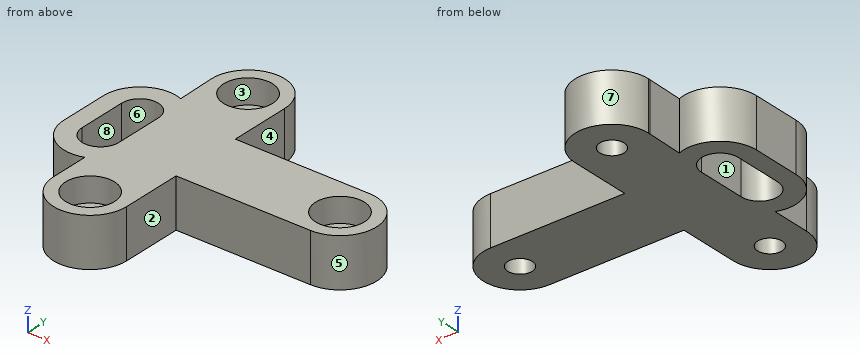
```python
from build123d import *

# Parameters (mm, degrees)
T_BRACKET_PLATE_20MM_DEPTH     = 20
POCKET_A_SKETCH_R              = 10
TRIANGULAR_POCKET_A_10MM_DEPTH = 10
POCKET_B_SKETCH_R              = 5
TRIANGULAR_POCKET_B_10MM_DEPTH = 10


with BuildPart() as part:
    # T Profile Sketch → T Bracket Plate 20mm (new body)
    with BuildSketch(Plane.XY):
        with BuildLine():
            ThreePointArc((-14.647668653, 24.012585384), (-28.506322055, 22.354856741), (-35, 10))
            Line((-35, 10), (-35, -10))
            ThreePointArc((-35, -10), (-28.660254038, -22.247448714), (-15, -24.142135624))
            Line((-15, -24.142135624), (-15, -40))
            ThreePointArc((-15, -40), (0, -55), (15, -40))
            Line((15, -40), (15, -15))
            Line((15, -15), (70, -15))
            ThreePointArc((70, -15), (85, 0), (70, 15))
            Line((70, 15), (15, 15))
            Line((15, 15), (15, 40))
            ThreePointArc((15, 40), (0, 55), (-15, 40))
            Line((-15, 40), (-14.985436811, 39.339179624))
            Line((-14.985436811, 39.339179624), (-14.647668653, 24.012585384))
        make_face()
        with BuildLine():
            Line((-27.5, -10), (-27.5, 10))
            ThreePointArc((-27.5, 10), (-20, 17.5), (-12.5, 10))
            Line((-12.5, 10), (-12.5, -10))
            ThreePointArc((-12.5, -10), (-20, -17.5), (-27.5, -10))
        make_face(mode=Mode.SUBTRACT)
    extrude(amount=T_BRACKET_PLATE_20MM_DEPTH)

    # Pocket A Sketch → Triangular Pocket A 10mm (cut)
    with BuildSketch(Plane.XY.offset(20)):
        with Locations((0, 40)):
            Circle(POCKET_A_SKETCH_R)
        with Locations((0, -40)):
            Circle(POCKET_A_SKETCH_R)
        with Locations((70, 0)):
            Circle(POCKET_A_SKETCH_R)
    extrude(amount=-TRIANGULAR_POCKET_A_10MM_DEPTH, mode=Mode.SUBTRACT)

    # Pocket B Sketch → Triangular Pocket B 10mm (cut)
    with BuildSketch(Plane.XY.offset(10)):
        with Locations((0, 40)):
            Circle(POCKET_B_SKETCH_R)
        with Locations((0, -40)):
            Circle(POCKET_B_SKETCH_R)
        with Locations((70, 0)):
            Circle(POCKET_B_SKETCH_R)
    extrude(amount=-TRIANGULAR_POCKET_B_10MM_DEPTH, mode=Mode.SUBTRACT)


solid = part.part
```
For this review, take the finished solid that the model builds, in its own axes (mm). Face numbers are marked on the shaded views. A direction names the side the tool comes from. Coordinates: 2 decimals unless noted, no trailing zeros. Loops run counter-clockwise (first coordinate to the right, second up) from the corner with the lowest first, then second, coordinate; pieces in that order, holes last.
1. Insertion check: P1, Ø11.5, axis at x = 0, y = 40, coming from the +Z side; P2, Ø5, axis at x = 55.5, z = 2, coming from the +Y side; P3, Ø4, axis at x = 38.5, z = 2.5, coming from the -Y side. Each pin has a flat end and moves straight along its axis. Give the tip position at first contact, or say it passes through.
2. For line 1 (Y direction, x = 0, z = 13.5); line 2 (X direction, y = 1.5, z = 10.5); line 3 (Y direction, x = 1.5, z = 17), list the stretches that pass through material, from the lowest coordinate up.
3. Mouldability with a two-part tool opening along Y and no side actions: class the marked faces 5, 6, 7 and 8 as +Y half, -Y half, draft (parallel to the pull), parting line (faces both ways), or undercut.
4. For the marked faces 1, 2, 3 and 4, list the 3-axis set-ups (+Z, -Z, +X, -X, +Y, -Y) from which the entire face can be reached by the end or side of a thin tool; tool diameter is ignored.
5. Add section C-C, the plane x = 0. Give the boundary of the cut face in (y, z), then the cut area to 3 significant figures.
6. Add section A-A, the plane x = -20. Give the boundary of the cut face in (y, z), then the cut area to 3 significant figures.
7. Add section B-B, the plane z = 7.5. Give the boundary of the cut face in (x, y), then the cut area to 3 significant figures.
8. Add section D-D, the plane y = 33. Give the boundary of the cut face in (x, z).
Result:
1. P1: stops at z = 10
1. P2: stops at y = 15
1. P3: stops at y = -15
2. line 1: y = -55 to -50, -30 to 30, 50 to 55
2. line 2: x = -35 to -27.5, -12.5 to 60.11, 79.89 to 84.92
2. line 3: y = -54.92 to -49.89, -30.11 to 30.11, 49.89 to 54.92
3. face 5: parting line
3. face 6: undercut
3. face 7: +Y half
3. face 8: undercut
4. face 1: +Z, -Z
4. face 2: +Z, -Z, +X, -Y
4. face 3: +Z
4. face 4: +Z, -Z, +X, +Y
5. outline: (-55, 0) - (-45, 0) - (-45, 10) - (-50, 10) - (-50, 20) - (-55, 20) - close; (-35, 0) - (35, 0) - (35, 10) - (30, 10) - (30, 20) - (-30, 20) - (-30, 10) - (-35, 10) - close; (45, 0) - (55, 0) - (55, 20) - (50, 20) - (50, 10) - (45, 10) - close
5. area: 1,600 mm2
6. outline: (-25, 0) - (-17.5, 0) - (-17.5, 20) - (-25, 20) - close; (17.5, 0) - (25, 0) - (25, 20) - (17.5, 20) - close
6. area: 300 mm2
7. outline: (-35, -10) arc R15 ccw to (-15, -24.14) - (-15, -40) arc R15 ccw to (15, -40) - (15, -15) - (70, -15) arc R15 ccw to (70, 15) - (15, 15) - (15, 40) arc R15 ccw to (-15, 40) - (-14.65, 24.01) arc R15 ccw to (-35, 10) - close; hole (-27.5, -10) arc R7.5 ccw to (-12.5, -10) - (-12.5, 10) arc R7.5 ccw to (-27.5, 10) - close; hole circle Ø10 at (0, -40); hole circle Ø10 at (0, 40); hole circle Ø10 at (70, 0)
7. area: 5,300 mm2
8. outline: (-14.85, 0) - (15, 0) - (15, 20) - (7.14, 20) - (7.14, 10) - (-7.14, 10) - (-7.14, 20) - (-14.85, 20) - close
